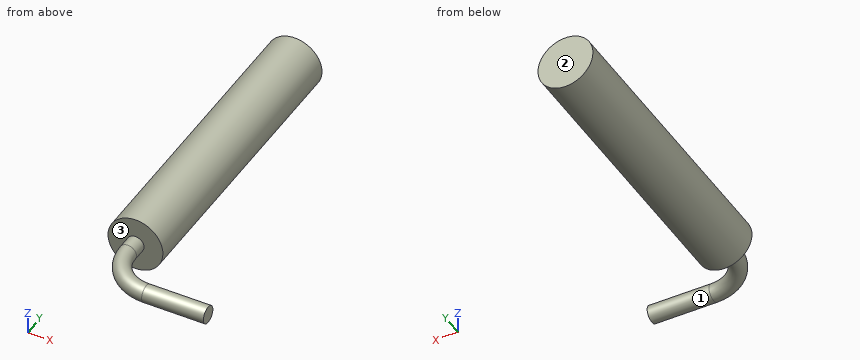
from build123d import *

# Parameters (mm, degrees)
SKETCH1_R           = 4
BOSS_EXTRUDE1_DEPTH = 42
SKETCH2_R           = 1.25


with BuildPart() as part:
    # Sketch1 → Boss-Extrude1 (new body)
    with BuildSketch(Plane(origin=(0, 0, 0), x_dir=(1, 0, 0), z_dir=(0, 1, 0))):
        with Locations(Location((0, 0, 0), (0, 0, 90))):
            Circle(SKETCH1_R)
    extrude(amount=BOSS_EXTRUDE1_DEPTH)

    # Sweep1: sweep along a path in Sketch3
    with BuildLine(Plane.XY) as sweep1_path:
        Line((0, 0), (0, -2))
        ThreePointArc((0, -2), (1.757359313, -6.242640687), (6, -8))
        Line((6, -8), (15, -8))
    # Sketch2 → Sweep1 (sweep)
    with BuildSketch(Plane.XZ):
        Circle(SKETCH2_R)
    sweep(path=sweep1_path.line)


solid = part.part
Geometry: final body of the model. Coordinates: model frame, mm. Face numbers are marked on the shaded views. A direction names the side the tool comes from. Round coordinates to 2 decimals unless told otherwise and drop trailing zeros. Order: outer loops, then holes, each group sorted by start corner. A loop starts at its lowest first (then second) coordinate and runs counter-clockwise, first axis right, second up.
Q1. Section B-B, the plane y = 31.5. Output: boundary loops of the cut face in (x, z), and give its area (3 significant figures).
Result sheet:
outline: circle Ø8 at (0, 0)
area: 50.3 mm2
Q2. Access query for the marked faces 1, 2 and 3. Directions: +Z, -Z, +X, -X, +Y, -Y. A direction counts if a zero-diameter tool reaches every point of the face in a straight line with its end or side. Return the directions, or none.
Result sheet:
face 1: +X
face 2: +Z, -Z, +X, -X, +Y
face 3: none
Q3. Pin query (flat end, axial travel): pin 1 (4 mm diameter, centred on y = 15.5, z = -2.5, fed in from +X); pin 2 (2 mm diameter, centred on x = 6, y = 26.5, fed in from -Z); pin 3 (1.5 mm diameter, centred on x = 7.5, z = 1.5, fed in from +Y); pin 4 (1 mm diameter, centred on y = 25.5, z = -2, fed in from -X). Return the tip coordinate at first contact, or that it passes through.
Result sheet:
pin 1: stops at x = 3.97
pin 2: passes through
pin 3: stops at y = -7
pin 4: stops at x = -3.71
Q4. Section C-C, the plane x = 12.75. Output: boundary loops of the cut face in (y, z).
Result sheet:
outline: circle Ø2.5 at (-8, 0)
Q5. Section A-A, the plane z = 0. Output: boundary loops of the cut face in (x, y).
Result sheet:
outline: (-4, 0) - (-1.25, 0) - (-1.25, -2) arc R7.25 ccw to (6, -9.25) - (15, -9.25) - (15, -6.75) - (6, -6.75) arc R4.75 cw to (1.25, -2) - (1.25, 0) - (4, 0) - (4, 42) - (-4, 42) - close
Q6. Section D-D, the plane z = -2.25. Output: boundary loops of the cut face in (x, y).
Result sheet:
outline: (-3.31, 0) - (3.31, 0) - (3.31, 42) - (-3.31, 42) - close
Q7. Material intervals for probe 1 along Y at (x, z) = (-0.5, -1.5); probe 2 along X at (y, z) = (12.5, -1.75); probe 3 along X at (y, z) = (-2, 1), sorted ascending.
Result sheet:
probe 1: y = 0 to 42
probe 2: x = -3.6 to 3.6
probe 3: x = -0.75 to 0.75
